Can you work these out from the model? Positions are in its coordinate system, mm. A direction names the side the tool comes from. Give positions to 0.01 mm unless a question says otherwise; leave off trailing zeros. Order: outer loops, then holes, each group sorted by start corner. A loop starts at its lowest first (then second) coordinate and runs counter-clockwise, first axis right, second up.
Item 1: If we mould it in two halves opening along X, with no side actions, what happens to faces 1 (the flat face through (7, 90, 1)), 2 (the flat face through (0, 47, -50)), 3 (the flat face through (18.5, 7, 0))? For each: +X half, -X half, draft (parallel to the pull), parting line (faces both ways), or undercut.
Item 2: I want a section at C-C, the plane z = 36.5. Write out the boundary of the cut face in (x, y), then the cut area to 3 significant figures.
Item 3: I'm going to push flat-ended pins straight in: pin 1 Ø3 at (x, y) = (-7.5, 76.5) entering from +Z; pin 2 Ø22.5 at (y, z) = (91, -21) entering from -X; pin 3 Ø5 at (x, z) = (13.5, -22.5) entering from +Y; pin 4 Ø12 at (y, z) = (113, 2.5) entering from +X. Where does each tip first touch, or does it pass through?
Item 4: I want a section at A-A, the plane z = -2.5. Write out the boundary of the cut face in (x, y), then the cut area to 4 significant figures.
Item 5: Which directions (+Z, -Z, +X, -X, +Y, -Y) give clear straight access to the entire face, cutting with the end or side of a thin tool? Please do faces 4 (the cylindrical face through (15.1, 7.1, 28.5)), 5 (the flat face through (5.5, 68, 1)), 6 (the flat face through (5.5, 112, 1)).
Item 6: I want a section at D-D, the plane y = 40. Write out the boundary of the cut face in (x, z), then the cut area to 3 significant figures.
Item 7: If I drill on line 1 along X through (y, z) = (12, 18.5); line 2 along X through (y, z) = (19, -21.5); line 3 along Y through (x, z) = (-13.5, -32), over which ranges is the centre line in solid material (lowest first)?
Item 8: I want a section at B-B, the plane x = 15.5. Write out the boundary of the cut face in (y, z).
```python
from build123d import *

# Parameters (mm, degrees)
EXTRUDE_1_DEPTH     = 50
CUT_EXTRUDE_1_REACH = 120.55
SKETCH_3_W          = 100
SKETCH_3_H          = 15
SKETCH_3_H_2        = 16
CUT_EXTRUDE_2_DEPTH = 1.5


with BuildPart() as part:
    # 草图1 → 凸台-拉伸1 (new, symmetric)
    with BuildSketch(Plane.XY):
        Polygon((0, 0), (23, 0), (23, 14), (7, 14), (7, 119), (-7, 119), (-7, 14), (-23, 14), (-23, 0), align=None)
    extrude(amount=EXTRUDE_1_DEPTH, both=True)

    # 草图2 → 切除-拉伸1 (cut, up to next)
    with BuildSketch(Plane(origin=(0, 14, 0), x_dir=(1, 0, 0), z_dir=(0, 1, 0)), mode=Mode.PRIVATE) as cut_extrude_1_sk1:
        with BuildLine():
            Line((11.5, -25), (11.5, 25))
            ThreePointArc((11.5, 25), (15, 28.5), (18.5, 25))
            Line((18.5, 25), (18.5, -25))
            ThreePointArc((18.5, -25), (15, -28.5), (11.5, -25))
        make_face()
    cut_extrude_1_tool1 = extrude(cut_extrude_1_sk1.sketch, amount=-CUT_EXTRUDE_1_REACH, mode=Mode.PRIVATE) & part.part
    cut_extrude_1 = cut_extrude_1_tool1.solids().sort_by_distance((15, 14, 0))[0]
    add(cut_extrude_1, mode=Mode.SUBTRACT)

    # 草图3 → 切除-拉伸2 (cut)
    with BuildSketch(Plane(origin=(7, 0, 0), x_dir=(0, 0, -1), z_dir=(1, 0, 0))):
        with Locations((0, 111.5)):
            Rectangle(SKETCH_3_W, SKETCH_3_H)
        with Locations((0, 68)):
            Rectangle(SKETCH_3_W, SKETCH_3_H_2)
    cut_extrude_2 = extrude(amount=-CUT_EXTRUDE_2_DEPTH, mode=Mode.SUBTRACT)

    # 镜向1: 切除-拉伸1 across plane
    add(cut_extrude_1.mirror(Plane(origin=(0, 0, 0), x_dir=(0, 0, 1), z_dir=(1, 0, 0))), mode=Mode.SUBTRACT)

    # 镜向2: 切除-拉伸2 across plane
    add(cut_extrude_2.mirror(Plane(origin=(0, 0, 0), x_dir=(0, 0, 1), z_dir=(1, 0, 0))), mode=Mode.SUBTRACT)


solid = part.part
```
Results list:
1. face 1: +X half
1. face 2: draft
1. face 3: undercut
2. outline: (-23, 0) - (23, 0) - (23, 14) - (7, 14) - (7, 60) - (5.5, 60) - (5.5, 76) - (7, 76) - (7, 104) - (5.5, 104) - (5.5, 119) - (-5.5, 119) - (-5.5, 104) - (-7, 104) - (-7, 76) - (-5.5, 76) - (-5.5, 60) - (-7, 60) - (-7, 14) - (-23, 14) - close
2. area: 2,020 mm2
3. pin 1: stops at z = 50
3. pin 2: stops at x = -7
3. pin 3: stops at y = 14
3. pin 4: stops at x = 5.5
4. outline: (-23, 0) - (-18.5, 0) - (-18.5, 14) - (-23, 14) - close; (-11.5, 0) - (11.5, 0) - (11.5, 14) - (7, 14) - (7, 60) - (5.5, 60) - (5.5, 76) - (7, 76) - (7, 104) - (5.5, 104) - (5.5, 119) - (-5.5, 119) - (-5.5, 104) - (-7, 104) - (-7, 76) - (-5.5, 76) - (-5.5, 60) - (-7, 60) - (-7, 14) - (-11.5, 14) - close; (18.5, 0) - (23, 0) - (23, 14) - (18.5, 14) - close
4. area: 1,825 mm2
5. face 4: +Y, -Y
5. face 5: +Z, -Z, +X
5. face 6: +Z, -Z, +X, +Y
6. outline: (-7, -50) - (7, -50) - (7, 50) - (-7, 50) - close
6. area: 1,400 mm2
7. line 1: x = -23 to -18.5, -11.5 to 11.5, 18.5 to 23
7. line 2: x = -7 to 7
7. line 3: y = 0 to 14
8. outline: (0, -50) - (14, -50) - (14, -28.46) - (0, -28.46) - close; (0, 28.46) - (14, 28.46) - (14, 50) - (0, 50) - close
